```python
from build123d import *

# Parameters (mm, degrees)
SKETCH1_W             = 34
SKETCH1_H             = 45
BOSS_EXTRUDE1_DEPTH   = 59
SKETCH2_W             = 25
SKETCH2_H             = 39
CUT_EXTRUDE1_DEPTH    = 45
CHAMFER1_SIZE         = 10
FILLET1_R             = 10
M5_TAPPED_HOLE1_D     = 4.2
M5_TAPPED_HOLE1_DEPTH = 12.4
M5_TAPPED_HOLE1_TIP   = 1.2618073
M5_TAPPED_HOLE2_D     = 4.2
M5_TAPPED_HOLE2_DEPTH = 12.4
M5_TAPPED_HOLE2_TIP   = 1.2618073


with BuildPart() as part:
    # Sketch1 → Boss-Extrude1 (new body)
    with BuildSketch(Plane(origin=(0, 0, 0), x_dir=(1, 0, 0), z_dir=(0, 1, 0))):
        Rectangle(SKETCH1_W, SKETCH1_H)
    extrude(amount=BOSS_EXTRUDE1_DEPTH)

    # Sketch2 → Cut-Extrude1 (cut)
    with BuildSketch(Plane(origin=(17, 0, 0), x_dir=(0, 0, -1), z_dir=(1, 0, 0))):
        with Locations((-10, 39.5)):
            Rectangle(SKETCH2_W, SKETCH2_H)
    extrude(amount=-CUT_EXTRUDE1_DEPTH, mode=Mode.SUBTRACT)

    # Chamfer1
    chamfer1_edges = [part.edges().sort_by_distance(p)[0] for p in [
        (0, 0, -22.5),
    ]]
    chamfer(chamfer1_edges, length=CHAMFER1_SIZE)

    # Fillet1
    fillet1_edges = [part.edges().sort_by_distance(p)[0] for p in [
        (0, 20, -2.5),
    ]]
    fillet(fillet1_edges, radius=FILLET1_R)

    # M5 Tapped Hole1
    with Locations(Plane(origin=(-11, 59, -12.5), x_dir=(0, 0, 1), z_dir=(0, 1, 0))):
        with Locations((0, 0), (0, 22)):
            Hole(M5_TAPPED_HOLE1_D / 2, depth=M5_TAPPED_HOLE1_DEPTH)
            with Locations((0, 0, -(M5_TAPPED_HOLE1_DEPTH + M5_TAPPED_HOLE1_TIP / 2))):  # 118° drill point
                Cone(0, M5_TAPPED_HOLE1_D / 2, M5_TAPPED_HOLE1_TIP, mode=Mode.SUBTRACT)

    # M5 Tapped Hole2
    with Locations(Plane(origin=(-12.5, 10, 22.5), x_dir=(1, 0, 0), z_dir=(0, 0, 1))):
        with Locations((0, 0), (25, 0)):
            Hole(M5_TAPPED_HOLE2_D / 2, depth=M5_TAPPED_HOLE2_DEPTH)
            with Locations((0, 0, -(M5_TAPPED_HOLE2_DEPTH + M5_TAPPED_HOLE2_TIP / 2))):  # 118° drill point
                Cone(0, M5_TAPPED_HOLE2_D / 2, M5_TAPPED_HOLE2_TIP, mode=Mode.SUBTRACT)


solid = part.part
```
Work out the finished part from the listing and answer in its coordinate system (mm). A direction names the side the tool comes from. Give positions to 0.01 mm unless a question says otherwise; leave off trailing zeros. Order: outer loops, then holes, each group sorted by start corner. A loop starts at its lowest first (then second) coordinate and runs counter-clockwise, first axis right, second up. Notation, with made-up numbers: (32, 81) - (49, 81) arc R16 cw to (49, 87) - close; hole circle Ø3 at (-20.75, -22.5). An arc over 180 degrees is marked (long way). One line per item, written item: value. Start each with the question number.
1. Section B-B, the plane z = 15.5 is taken. Write down the section's boundary in (x, y), then the cut area to 3 significant figures.
2. Consider line 1 (X direction, y = 54, z = -12.5); line 2 (X direction, y = 10, z = 17.25); line 3 (Y direction, x = -12.5, z = 13). Determine where each line is inside the solid, lowest interval first.
3. Section C-C, the plane x = 0 is taken. Write down the section's boundary in (y, z), then the cut area to 3 significant figures.
4. Section D-D, the plane y = 39 is taken. Write down the section's boundary in (x, z).
5. Each of these flat-tipped pins is pushed along its axis until it touches: pin 1 Ø16.5 at (x, z) = (-5.5, 13) entering from +Y; pin 2 Ø1 at (x, y) = (-12, 51) entering from +Z; pin 3 Ø2 at (x, z) = (-7.5, 12.5) entering from +Y. Where does it stop, or does it pass through?
6. For a pull along Y with two mould halves and no side action, classify faces 1 (the face through (11.09, 52.71, -10.4)), 2 (the face through (-0.2, 5.1, -17.6)), 3 (the face through (-12.227, 12.082, 16.213)) as released by +Y, released by -Y, zero draft, split by the parting line, or undercut.
7. Section A-A, the plane y = 52.5 is taken. Write down the section's boundary in (x, z).
8. Which of the six approach directions +Z, -Z, +X, -X, +Y, -Y give full straight-line access (tool end or side, diameter ignored) to faces 4 (the face through (-8.918, 52.713, -12.227)), 5 (the face through (0, 44, -2.5)), 6 (the face through (12.773, 12.082, 16.213))?
Filled sheet:
1. outline: (-17, 0) - (17, 0) - (17, 20) - (-17, 20) - close; hole circle Ø4.2 at (-12.5, 10); hole circle Ø4.2 at (12.5, 10)
1. area: 652 mm²
2. line 1: -17 to -13.1, -8.9 to 8.9, 13.1 to 17
2. line 2: -17 to -14.6, -10.4 to 10.4, 14.6 to 17
2. line 3: 0 to 7.9, 12.1 to 20
3. outline: (0, -12.5) - (10, -22.5) - (59, -22.5) - (59, -2.5) - (30, -2.5) arc R10 cw to (20, 7.5) - (20, 22.5) - (0, 22.5) - close
3. area: 1,650 mm²
4. outline: (-17, -22.5) - (17, -22.5) - (17, -2.5) - (-17, -2.5) - close
5. pin 1: y = 20.39
5. pin 2: z = -2.5
5. pin 3: y = 20
6. face 1: zero draft
6. face 2: released by -Y
6. face 3: undercut
7. outline: (-17, -22.5) - (17, -22.5) - (17, -2.5) - (-17, -2.5) - close; hole circle Ø4.2 at (-11, -12.5); hole circle Ø4.2 at (11, -12.5)
8. face 4: +Y
8. face 5: +Z, +X, -X, +Y
8. face 6: +Z
